Could you check a few things on this drawing? It's one solid part, dimensions in mm from its lowest x, y, z. A direction names the side the tool comes from. Coordinates: 2 decimals unless noted, no trailing zeros. Write each loop counter-clockwise with the first axis right and the second up, starting at its lowest first coordinate (ties: lowest second). Pieces come first, ordered by that corner, then holes. Notation, with made-up numbers: (89, 12.25) - (97, 12.25) arc R14 cw to (97, 29.25) - close; hole circle Ø7 at (-28.5, 83). An arc over 180 degrees is marked (long way). Answer as a JSON object with one key per item and string values. Group by question number.
1) On a 3-axis mill with a long thin cutter (end or side, diameter ignored), from which of +Z, -Z, +X, -X, +Y, -Y can I reach the whole of each face in a straight line? I mean the marked faces 1 and 2. Say none if no direction works.
2) Please list where these lines run through material, in increasing order: line 1 along Y through (x, z) = (15, 1.5); line 2 along Y through (x, z) = (10.5, 17.25); line 3 along Z through (x, y) = (25, 1.1).
3) If we section it at D-D (z = 1.5): Write out the boundary of the cut face in (x, y), plus the area to 3 significant figures.
4) If we section it at B-B (y = 10.5): Write out the boundary of the cut face in (x, z), plus the area to 3 significant figures.
5) If we section it at C-C (x = 5): Write out the boundary of the cut face in (y, z), plus the area to 3 significant figures.
6) We'd pull the mould along Y, two halves only. Please class the marked faces 3, 4, 5 and 6: released by +Y, released by -Y, zero draft, split by the parting line, or undercut.
7) If we section it at A-A (z = 12): Write out the boundary of the cut face in (x, y), plus the area to 3 significant figures.
8) Will this pin go through, and if not, where does the flat tip stop? pin 1 Ø13.5 at (x, y) = (9.5, 14) entering from +Z.
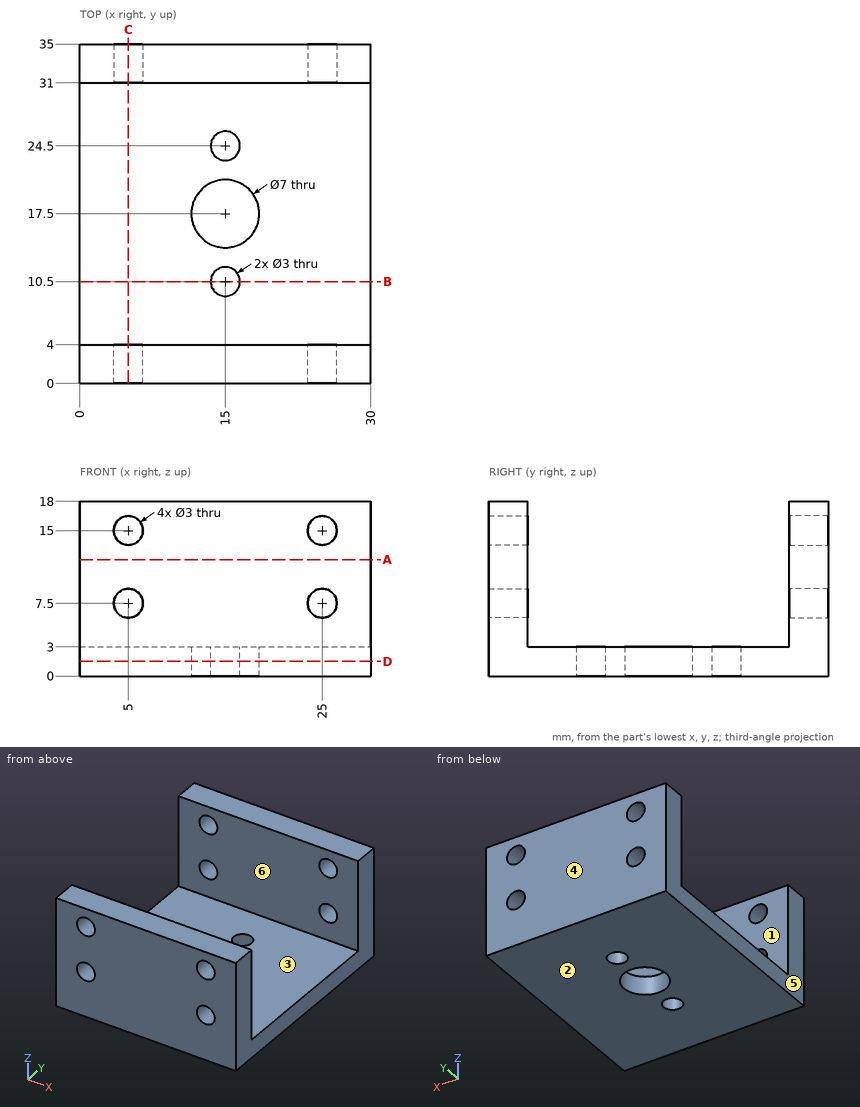
Here are the results:
{
 "1": {"face 1": "+Z, +X, -X", "face 2": "-Z, +X, -X, +Y, -Y"},
 "2": {"line 1": "y = 0 to 9, 12 to 14, 21 to 23, 26 to 35", "line 2": "y = 0 to 4, 31 to 35", "line 3": "z = 0 to 6, 9 to 13.5, 16.5 to 18"},
 "3": {"outline": "(0, 0) - (30, 0) - (30, 35) - (0, 35) - close; hole circle Ø7 at (15, 17.5); hole circle Ø3 at (15, 10.5); hole circle Ø3 at (15, 24.5)", "area": "997 mm²"},
 "4": {"outline": "(0, 0) - (13.5, 0) - (13.5, 3) - (0, 3) - close; (16.5, 0) - (30, 0) - (30, 3) - (16.5, 3) - close", "area": "81.0 mm²"},
 "5": {"outline": "(0, 0) - (35, 0) - (35, 6) - (31, 6) - (31, 3) - (4, 3) - (4, 6) - (0, 6) - close; (0, 9) - (4, 9) - (4, 13.5) - (0, 13.5) - close; (0, 16.5) - (4, 16.5) - (4, 18) - (0, 18) - close; (31, 9) - (35, 9) - (35, 13.5) - (31, 13.5) - close; (31, 16.5) - (35, 16.5) - (35, 18) - (31, 18) - close", "area": "177 mm²"},
 "6": {"face 3": "undercut", "face 4": "released by +Y", "face 5": "zero draft", "face 6": "undercut"},
 "7": {"outline": "(0, 0) - (30, 0) - (30, 4) - (0, 4) - close; (0, 31) - (30, 31) - (30, 35) - (0, 35) - close", "area": "240 mm²"},
 "8": {"pin 1": "stops at z = 3"}
}
